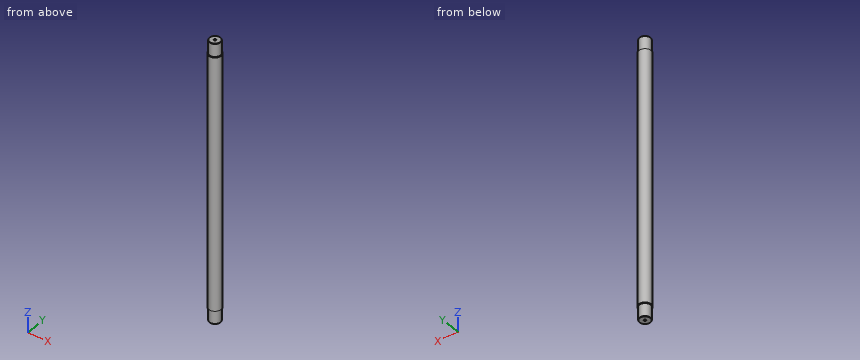
from build123d import *

# Parameters (mm, degrees)
SKETCH_1_R              = 22.5
EXTRUDE_1_DEPTH         = 904.6
SKETCH_2_R              = 20
EXTRUDE_2_DEPTH         = 47.7
EXTRUDE_START           = 47.7
SKETCH_3_R              = 20
EXTRUDE_3_DEPTH         = 47.7
FILLET_1_R              = 1
CHAMFER_1_SIZE          = 1
HOLE_WIZARD_M10_1_D     = 8.5
HOLE_WIZARD_M10_1_DEPTH = 24.5
HOLE_WIZARD_M10_1_TIP   = 2.553657631
HOLE_WIZARD_M10_2_D     = 8.5
HOLE_WIZARD_M10_2_DEPTH = 24.5
HOLE_WIZARD_M10_2_TIP   = 2.553657631


with BuildPart() as part:
    # 草图1 → 凸台-拉伸1 (new body)
    with BuildSketch(Plane.XY):
        with Locations(Location((0, 0, 0), (0, 0, 180))):
            Circle(SKETCH_1_R)
    extrude(amount=EXTRUDE_1_DEPTH)

    # 草图2 → 凸台-拉伸2 (add)
    with BuildSketch(Plane.XY.offset(904.6)):
        Circle(SKETCH_2_R)
    extrude(amount=EXTRUDE_2_DEPTH)

    # 草图3 → 凸台-拉伸3 (add)
    with BuildSketch(Plane(origin=(0, 0, 0), x_dir=(-1, 0, 0), z_dir=(0, 0, -1)).offset(EXTRUDE_START)):
        with Locations(Location((0, 0, 0), (0, 0, 180))):
            Circle(SKETCH_3_R)
    extrude(amount=-EXTRUDE_3_DEPTH)

    # 圆角1
    fillet_1_edges = [part.edges().sort_by_distance(p)[0] for p in [
        (-20, 0, 904.6),
        (-20, 0, 0),
    ]]
    fillet(fillet_1_edges, radius=FILLET_1_R)

    # 倒角1
    chamfer_1_edges = [part.edges().sort_by_distance(p)[0] for p in [
        (-20, 0, -47.7),
        (-20, 0, 952.3),
    ]]
    chamfer(chamfer_1_edges, length=CHAMFER_1_SIZE)

    # M10 螺纹孔1
    with Locations(Plane.XY.offset(952.3)):
        with Locations((0, 0)):
            Hole(HOLE_WIZARD_M10_1_D / 2, depth=HOLE_WIZARD_M10_1_DEPTH)
            with Locations((0, 0, -(HOLE_WIZARD_M10_1_DEPTH + HOLE_WIZARD_M10_1_TIP / 2))):  # 118° drill point
                Cone(0, HOLE_WIZARD_M10_1_D / 2, HOLE_WIZARD_M10_1_TIP, mode=Mode.SUBTRACT)

    # M10 螺纹孔2
    with Locations(Plane(origin=(0, 0, -47.7), x_dir=(-1, 0, 0), z_dir=(0, 0, -1))):
        with Locations((0, 0)):
            Hole(HOLE_WIZARD_M10_2_D / 2, depth=HOLE_WIZARD_M10_2_DEPTH)
            with Locations((0, 0, -(HOLE_WIZARD_M10_2_DEPTH + HOLE_WIZARD_M10_2_TIP / 2))):  # 118° drill point
                Cone(0, HOLE_WIZARD_M10_2_D / 2, HOLE_WIZARD_M10_2_TIP, mode=Mode.SUBTRACT)


solid = part.part
Part model, mm, in its own coordinate system. Give positions to 0.01 mm unless a question says otherwise; leave off trailing zeros. Order: outer loops, then holes, each group sorted by start corner. A loop starts at its lowest first (then second) coordinate and runs counter-clockwise, first axis right, second up. Notation, with made-up numbers: (66.5, 58.25) - (92.5, 58.25) arc R33 ccw to (92.5, 96.25) - close; hole circle Ø1 at (19.5, -33.75). An arc over 180 degrees is marked (long way). One line per question, with ' | ' between items.
1. Drill centre lines: probe 1 along Y at (x, z) = (0, -36); probe 2 along Z at (x, y) = (15.5, 16); probe 3 along Y at (x, z) = (-2, 275). Where is each one in solid material? Low to high.
Filled in:
probe 1: -20 to -4.25, 4.25 to 20 | probe 2: 0 to 904.6 | probe 3: -22.41 to 22.41
2. Drop flat-ended pins along their axis: P1, Ø3, axis at y = 15, z = 475, coming from the +X side; P2, Ø1.5, axis at x = 13, z = 539.5, coming from the -Y side; P3, Ø5, axis at x = -11, z = 188, coming from the +Y side. Give the stop position or say it passes through.
Filled in:
P1: x = 18 | P2: y = -18.87 | P3: y = 20.83
3. Band-saw the part on A-A on z = 652.5. List the corners of the cut face in (x, y), then the cut area to 3 significant figures.
Filled in:
outline: circle Ø45 at (0, 0) | area: 1,590 mm²
